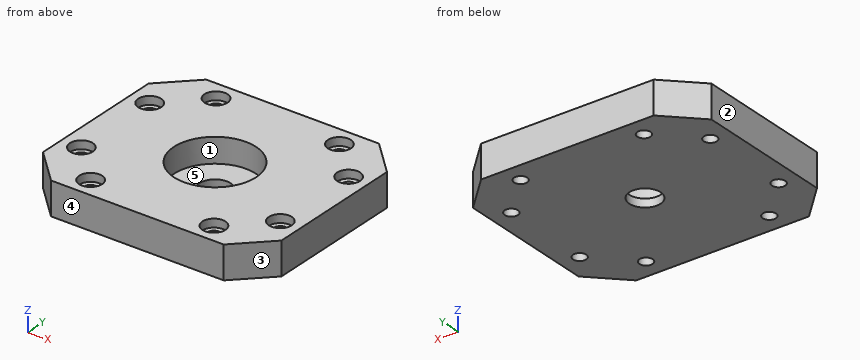
from build123d import *

# Parameters (mm, degrees)
SKETCH_1_W          = 145
SKETCH_1_H          = 125
EXTRUDE_1_DEPTH     = 20
CHAMFER_1_SIZE      = 20
SKETCH_2_R          = 7
CUT_EXTRUDE_1_DEPTH = 5
CUT_EXTRUDE_2_REACH = 98.889
SKETCH_3_R          = 4
CUT_EXTRUDE_5_REACH = 99.788
SKETCH_6_R          = 9.5
SKETCH_7_R          = 25
CUT_EXTRUDE_6_DEPTH = 15


with BuildPart() as part:
    # 草图1 → 凸台-拉伸1 (new body)
    with BuildSketch(Plane.XY):
        Rectangle(SKETCH_1_W, SKETCH_1_H)
    extrude(amount=EXTRUDE_1_DEPTH)

    # 倒角1
    chamfer_1_edges = [part.edges().sort_by_distance(p)[0] for p in [
        (72.5, -62.5, 10),
        (-72.5, -62.5, 10),
        (-72.5, 62.5, 10),
        (72.5, 62.5, 10),
    ]]
    chamfer(chamfer_1_edges, length=CHAMFER_1_SIZE)

    # 草图2 → 切除-拉伸1 (cut)
    with BuildSketch(Plane.XY.offset(20)):
        with Locations((-37.5, 50.5)):
            Circle(SKETCH_2_R)
        with Locations((37.5, 50.5)):
            Circle(SKETCH_2_R)
        with Locations((-60.5, 27.5)):
            Circle(SKETCH_2_R)
        with Locations((-60.5, -27.5)):
            Circle(SKETCH_2_R)
        with Locations((-37.5, -50.5)):
            Circle(SKETCH_2_R)
        with Locations((37.5, -50.5)):
            Circle(SKETCH_2_R)
        with Locations((60.5, 27.5)):
            Circle(SKETCH_2_R)
        with Locations((60.5, -27.5)):
            Circle(SKETCH_2_R)
    extrude(amount=-CUT_EXTRUDE_1_DEPTH, mode=Mode.SUBTRACT)

    # 草图3 → 切除-拉伸2 (cut, up to next)
    with BuildSketch(Plane.XY.offset(15), mode=Mode.PRIVATE) as cut_extrude_2_sk1:
        with Locations((-37.5, 50.5)):
            Circle(SKETCH_3_R)
    cut_extrude_2_tool1 = extrude(cut_extrude_2_sk1.sketch, amount=-CUT_EXTRUDE_2_REACH, mode=Mode.PRIVATE) & part.part
    # 草图3 → 切除-拉伸2 (cut, up to next)
    with BuildSketch(Plane.XY.offset(15), mode=Mode.PRIVATE) as cut_extrude_2_sk2:
        with Locations((-60.5, 27.5)):
            Circle(SKETCH_3_R)
    cut_extrude_2_tool2 = extrude(cut_extrude_2_sk2.sketch, amount=-CUT_EXTRUDE_2_REACH, mode=Mode.PRIVATE) & part.part
    # 草图3 → 切除-拉伸2 (cut, up to next)
    with BuildSketch(Plane.XY.offset(15), mode=Mode.PRIVATE) as cut_extrude_2_sk3:
        with Locations((-60.5, -27.5)):
            Circle(SKETCH_3_R)
    cut_extrude_2_tool3 = extrude(cut_extrude_2_sk3.sketch, amount=-CUT_EXTRUDE_2_REACH, mode=Mode.PRIVATE) & part.part
    # 草图3 → 切除-拉伸2 (cut, up to next)
    with BuildSketch(Plane.XY.offset(15), mode=Mode.PRIVATE) as cut_extrude_2_sk4:
        with Locations((-37.5, -50.5)):
            Circle(SKETCH_3_R)
    cut_extrude_2_tool4 = extrude(cut_extrude_2_sk4.sketch, amount=-CUT_EXTRUDE_2_REACH, mode=Mode.PRIVATE) & part.part
    # 草图3 → 切除-拉伸2 (cut, up to next)
    with BuildSketch(Plane.XY.offset(15), mode=Mode.PRIVATE) as cut_extrude_2_sk5:
        with Locations((37.5, 50.5)):
            Circle(SKETCH_3_R)
    cut_extrude_2_tool5 = extrude(cut_extrude_2_sk5.sketch, amount=-CUT_EXTRUDE_2_REACH, mode=Mode.PRIVATE) & part.part
    # 草图3 → 切除-拉伸2 (cut, up to next)
    with BuildSketch(Plane.XY.offset(15), mode=Mode.PRIVATE) as cut_extrude_2_sk6:
        with Locations((60.5, 27.5)):
            Circle(SKETCH_3_R)
    cut_extrude_2_tool6 = extrude(cut_extrude_2_sk6.sketch, amount=-CUT_EXTRUDE_2_REACH, mode=Mode.PRIVATE) & part.part
    # 草图3 → 切除-拉伸2 (cut, up to next)
    with BuildSketch(Plane.XY.offset(15), mode=Mode.PRIVATE) as cut_extrude_2_sk7:
        with Locations((60.5, -27.5)):
            Circle(SKETCH_3_R)
    cut_extrude_2_tool7 = extrude(cut_extrude_2_sk7.sketch, amount=-CUT_EXTRUDE_2_REACH, mode=Mode.PRIVATE) & part.part
    # 草图3 → 切除-拉伸2 (cut, up to next)
    with BuildSketch(Plane.XY.offset(15), mode=Mode.PRIVATE) as cut_extrude_2_sk8:
        with Locations((37.5, -50.5)):
            Circle(SKETCH_3_R)
    cut_extrude_2_tool8 = extrude(cut_extrude_2_sk8.sketch, amount=-CUT_EXTRUDE_2_REACH, mode=Mode.PRIVATE) & part.part
    add(cut_extrude_2_tool1.solids().sort_by_distance((-37.5, 50.5, 15))[0], mode=Mode.SUBTRACT)
    add(cut_extrude_2_tool2.solids().sort_by_distance((-60.5, 27.5, 15))[0], mode=Mode.SUBTRACT)
    add(cut_extrude_2_tool3.solids().sort_by_distance((-60.5, -27.5, 15))[0], mode=Mode.SUBTRACT)
    add(cut_extrude_2_tool4.solids().sort_by_distance((-37.5, -50.5, 15))[0], mode=Mode.SUBTRACT)
    add(cut_extrude_2_tool5.solids().sort_by_distance((37.5, 50.5, 15))[0], mode=Mode.SUBTRACT)
    add(cut_extrude_2_tool6.solids().sort_by_distance((60.5, 27.5, 15))[0], mode=Mode.SUBTRACT)
    add(cut_extrude_2_tool7.solids().sort_by_distance((60.5, -27.5, 15))[0], mode=Mode.SUBTRACT)
    add(cut_extrude_2_tool8.solids().sort_by_distance((37.5, -50.5, 15))[0], mode=Mode.SUBTRACT)

    # 草图6 → 切除-拉伸5 (cut, up to next)
    with BuildSketch(Plane(origin=(0, 0, 0), x_dir=(-1, 0, 0), z_dir=(0, 0, -1)), mode=Mode.PRIVATE) as cut_extrude_5_sk1:
        Circle(SKETCH_6_R)
    cut_extrude_5_tool1 = extrude(cut_extrude_5_sk1.sketch, amount=-CUT_EXTRUDE_5_REACH, mode=Mode.PRIVATE) & part.part
    add(cut_extrude_5_tool1.solids().sort_by_distance((0, 0, 0))[0], mode=Mode.SUBTRACT)

    # 草图7 → 切除-拉伸6 (cut)
    with BuildSketch(Plane.XY.offset(20)):
        Circle(SKETCH_7_R)
    extrude(amount=-CUT_EXTRUDE_6_DEPTH, mode=Mode.SUBTRACT)


solid = part.part
The model under review builds one solid part; all positions refer to its coordinate system, in mm. Face numbers are marked on the shaded views. A direction names the side the tool comes from. Round coordinates to 2 decimals unless told otherwise and drop trailing zeros. Write each loop counter-clockwise with the first axis right and the second up, starting at its lowest first coordinate (ties: lowest second). Pieces come first, ordered by that corner, then holes. Notation, with made-up numbers: (84.5, 29.5) - (92.5, 29.5) arc R25 ccw to (92.5, 42.5) - close; hole circle Ø10 at (9.5, 0). An arc over 180 degrees is marked (long way). One line per item, written item: value. Start each with the question number.
1. Consider section A-A on y = -50.5. Write out the cut boundary in (x, z), and give its area (3 significant figures).
2. Machinability: for the marked faces 4 and 5, which of the approach directions +Z, -Z, +X, -X, +Y, -Y give a long, thin tool a straight path to every point of the face, cutting with its end or side? Answer none if there is none.
3. Clearance check with flat-ended pins moving along their axes: P1, Ø4, axis at x = 34.5, y = 49, coming from the +Z side; P2, Ø12, axis at x = 13.5, y = 10, coming from the +Z side. State where each tip first meets the part, or that it passes through.
4. Consider section B-B on z = 2. State how many separate pieces and enclosed holes the cut face has, and give its area (3 significant figures).
5. To check wall thickness, follow L1, parallel to Y at x = -37.5, z = 5; L2, parallel to Y at x = 60.5, z = 16.65; L3, parallel to X at y = 47.5, z = 17.75. State the ranges of each line that lie inside material, in increasing order. Write a range as from..to.
6. Consider section D-D on x = 0. Write out the cut boundary in (y, z).
7. Consider section C-C on x = 37.5. Write out the cut boundary in (y, z).
8. The part is to be moulded in two halves that separate along X. For the marked faces 1, 2 and 3, say which applies: released by +X, released by -X, zero draft, split by the parting line, or undercut.
Checks:
1. outline: (-64.5, 0) - (-41.5, 0) - (-41.5, 15) - (-44.5, 15) - (-44.5, 20) - (-64.5, 20) - close; (-33.5, 0) - (33.5, 0) - (33.5, 15) - (30.5, 15) - (30.5, 20) - (-30.5, 20) - (-30.5, 15) - (-33.5, 15) - close; (41.5, 0) - (64.5, 0) - (64.5, 20) - (44.5, 20) - (44.5, 15) - (41.5, 15) - close
1. area: 2,200 mm^2
2. face 4: +Z, -Z, +X, -X, -Y
2. face 5: +Z
3. P1: stops at z = 15
3. P2: stops at z = 5
4. separate pieces: 1
4. enclosed holes: 9
4. area: 16,600 mm^2
5. L1: y = -62.5..-54.5, -46.5..46.5, 54.5..62.5
5. L2: y = -54.5..-34.5, -20.5..20.5, 34.5..54.5
5. L3: x = -67.5..-43.82, -31.18..31.18, 43.82..67.5
6. outline: (-62.5, 0) - (-9.5, 0) - (-9.5, 5) - (-25, 5) - (-25, 20) - (-62.5, 20) - close; (9.5, 0) - (62.5, 0) - (62.5, 20) - (25, 20) - (25, 5) - (9.5, 5) - close
7. outline: (-62.5, 0) - (-54.5, 0) - (-54.5, 15) - (-57.5, 15) - (-57.5, 20) - (-62.5, 20) - close; (-46.5, 0) - (46.5, 0) - (46.5, 15) - (43.5, 15) - (43.5, 20) - (-43.5, 20) - (-43.5, 15) - (-46.5, 15) - close; (54.5, 0) - (62.5, 0) - (62.5, 20) - (57.5, 20) - (57.5, 15) - (54.5, 15) - close
8. face 1: undercut
8. face 2: released by -X
8. face 3: released by +X
